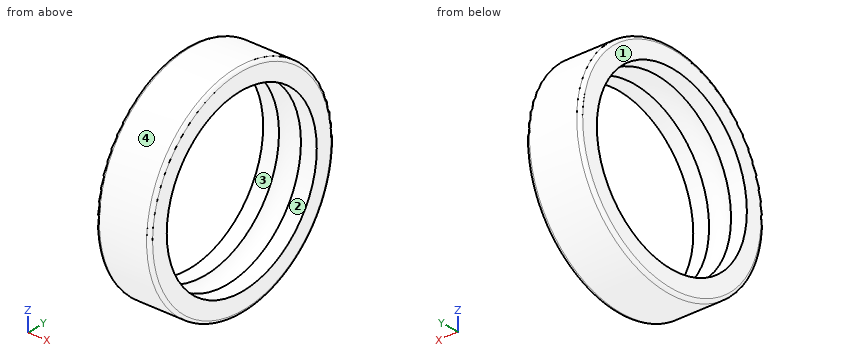
from build123d import *

# Parameters (mm, degrees)
FILLET1_R = 1.5


with BuildPart() as part:
    # Sketch1 → Revolve1 (revolve)
    with BuildSketch(Plane.XY, mode=Mode.PRIVATE) as revolve1_sk:
        with BuildLine():
            Line((5.120546846, 40.8), (12.5, 40.8))
            Line((12.5, 40.8), (12.5, 50))
            Line((12.5, 50), (-12.5, 50))
            Line((-12.5, 50), (-12.5, 40.8))
            Line((-12.5, 40.8), (-5.120546846, 40.8))
            ThreePointArc((-5.120546846, 40.8), (0, 43.1), (5.120546846, 40.8))
        make_face()
    revolve(revolve1_sk.sketch.rotate(Axis((-5.850943074, 0, 0), (1, 0, 0)), 90), axis=Axis((-5.850943074, 0, 0), (1, 0, 0)))

    # Fillet1
    fillet1_edges = [part.edges().sort_by_distance(p)[0] for p in [
        (-12.5, 0, -50),
        (12.5, 0, -50),
    ]]
    fillet(fillet1_edges, radius=FILLET1_R)


solid = part.part
Build history of the part. All positions in model axes, mm. Face numbers are marked on the shaded views. Coordinates: 2 decimals unless noted, no trailing zeros. Order: outer loops, then holes, each group sorted by start corner. A loop starts at its lowest first (then second) coordinate and runs counter-clockwise, first axis right, second up. Notation, with made-up numbers: (-11, 13.5) - (17, 13.5) arc R27 cw to (17, 50.5) - close; hole circle Ø6 at (89.25, 84). An arc over 180 degrees is marked (long way). Write each question's results on one line, items separated by ' | '. Start each with the question number.
Item 1: Flat gauge pins, fed straight in: pin 1 (8 mm diameter, centred on x = -6, z = 1, fed in from -Y); pin 2 (10 mm diameter, centred on x = -6, z = -38, fed in from +Y); pin 3 (8 mm diameter, centred on x = -4, y = -25.5, fed in from -Z). Where does each tip first touch, or does it go through?
Item 2: Wall check: probe 1 along Y at (x, z) = (7.75, 0); probe 2 along Y at (x, z) = (-11, -4); probe 3 along Z at (x, y) = (11, -15). Give the ranges that are in metal, low to high. Write a range as [from, to].
Item 3: Band-saw the part on C-C on x = -8.5. Write the cut outline in (y, z).
Item 4: Band-saw the part on A-A on z = 0. Write the cut outline in (x, y).
Item 5: Mould opens along Z. For the marked faces 1, 2, 3 and 4 say: released by +Z, released by -Z, zero draft, split by the parting line, or undercut.
Numbers:
1) pin 1: y = -50 | pin 2: y = 37.56 | pin 3: z = -45.14
2) probe 1: [-50, -40.8], [40.8, 50] | probe 2: [-49.84, -40.6], [40.6, 49.84] | probe 3: [-47.7, -37.94], [37.94, 47.7]
3) outline: circle Ø100 at (0, 0); hole circle Ø81.6 at (0, 0)
4) outline: (-12.5, -48.5) arc R1.5 ccw to (-11, -50) - (11, -50) arc R1.5 ccw to (12.5, -48.5) - (12.5, -40.8) - (5.12, -40.8) arc R6.85 cw to (-5.12, -40.8) - (-12.5, -40.8) - close; (-12.5, 40.8) - (-5.12, 40.8) arc R6.85 cw to (5.12, 40.8) - (12.5, 40.8) - (12.5, 48.5) arc R1.5 ccw to (11, 50) - (-11, 50) arc R1.5 ccw to (-12.5, 48.5) - close
5) face 1: zero draft | face 2: undercut | face 3: undercut | face 4: split by the parting line
